Read the model definition and answer for the solid it produces. Units are mm, in the model's axes. Give positions to 0.01 mm unless a question says otherwise; leave off trailing zeros. Write each loop counter-clockwise with the first axis right and the second up, starting at its lowest first coordinate (ties: lowest second). Pieces come first, ordered by that corner, then holes. Notation, with made-up numbers: M 18,62.5 L 29,62.5 A20 ccw 29,73.5 Z; hole C 56,61 d2. An arc over 180 degrees is marked long. Answer as CSV lines item,"result". Start each with the question number.
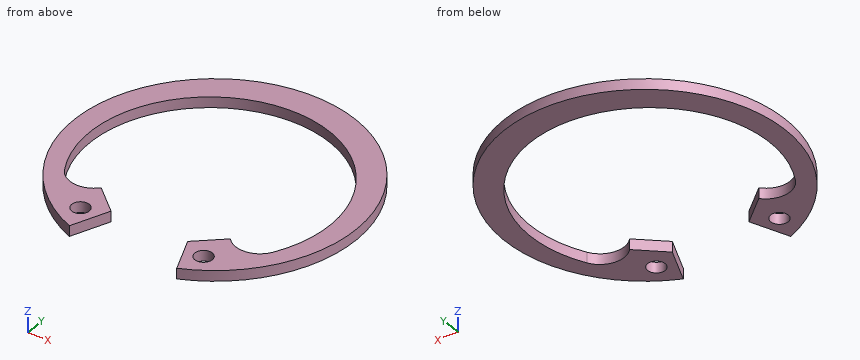
```python
from build123d import *

# Parameters (mm, degrees)
EXTRUDE_947_DEPTH      = 0.6
EXTRUDE_947_DEPTH_BACK = 0.6
SKETCH_1_R             = 1


with BuildPart() as part:
    # 草图1 → Extrude 947 (new, two sides: drawn at the far end of the back side and taken through both)
    with BuildSketch(Plane.XY.offset(-EXTRUDE_947_DEPTH_BACK)):
        with BuildLine():
            Line((-7.380473645, -7.931250769), (-4.381725301, -10.578420647))
            Line((-4.381725301, -10.578420647), (-6.142069089, -14.828266497))
            ThreePointArc((-6.142069089, -14.828266497), (0, 16.05), (6.142069089, -14.828266497))
            Line((6.142069089, -14.828266497), (4.381725301, -10.578420647))
            Line((4.381725301, -10.578420647), (7.380473645, -7.931250769))
            ThreePointArc((7.380473645, -7.931250769), (9.780239262, -8.8620448), (11.925945225, -7.440356203))
            ThreePointArc((11.925945225, -7.440356203), (0, 12.85), (-11.925945225, -7.440356203))
            ThreePointArc((-11.925945225, -7.440356203), (-9.780239262, -8.8620448), (-7.380473645, -7.931250769))
        make_face()
        with Locations((-7.034355028, -11.756183451)):
            Circle(SKETCH_1_R, mode=Mode.SUBTRACT)
        with Locations(Location((7.034355028, -11.756183451, 0), (0, 0, 180))):
            Circle(SKETCH_1_R, mode=Mode.SUBTRACT)
    extrude(amount=EXTRUDE_947_DEPTH + EXTRUDE_947_DEPTH_BACK)


solid = part.part
```
1. Given pin 1 (1.2 mm diameter, centred on x = 7.03, y = -11.76, fed in from +Z), flat-ended and moving along its own axis, determine where the tip first touches the part or whether it passes through.
2. Find section A-A on y = -1. Determine the outline of the cut face in (x, z).
3. Find section C-C on y = 9. Determine the outline of the cut face in (x, z), then the cut area to 3 significant figures.
4. Find section D-D on x = 0. Determine the outline of the cut face in (y, z), then the cut area to 3 significant figures.
5. Find the intervals of material crossed by line 1 (X direction, y = -11, z = 0.25); line 2 (Y direction, x = 0, z = 0.2); line 3 (X direction, y = -13, z = 0.3), in increasing order. Write a range as [from, to].
6. Find section B-B on z = -0.15. Determine the outline of the cut face in (x, y).
Computed:
1,pin 1,"passes through"
2,outline,"M -16.02,-0.6 L -13.65,-0.6 L -13.65,0.6 L -16.02,0.6 Z; M 13.65,-0.6 L 16.02,-0.6 L 16.02,0.6 L 13.65,0.6 Z"
3,outline,"M -13.29,-0.6 L -9.5,-0.6 L -9.5,0.6 L -13.29,0.6 Z; M 9.5,-0.6 L 13.29,-0.6 L 13.29,0.6 L 9.5,0.6 Z"
3,area,"9.09 mm^2"
4,outline,"M 12.85,-0.6 L 16.05,-0.6 L 16.05,0.6 L 12.85,0.6 Z"
4,area,"3.84 mm^2"
5,line 1,"x = [-11.69, -7.69], [-6.38, -4.56], [4.56, 6.38], [7.69, 11.69]"
5,line 2,"y = [12.85, 16.05]"
5,line 3,"x = [-9.41, -5.38], [5.38, 9.41]"
6,outline,"M -11.93,-7.44 A13.65 cw long 11.93,-7.44 A2.8 cw 7.38,-7.93 L 4.38,-10.58 L 6.14,-14.83 A16.05 ccw long -6.14,-14.83 L -4.38,-10.58 L -7.38,-7.93 A2.8 cw Z; hole C -7.03,-11.76 d2; hole C 7.03,-11.76 d2"
